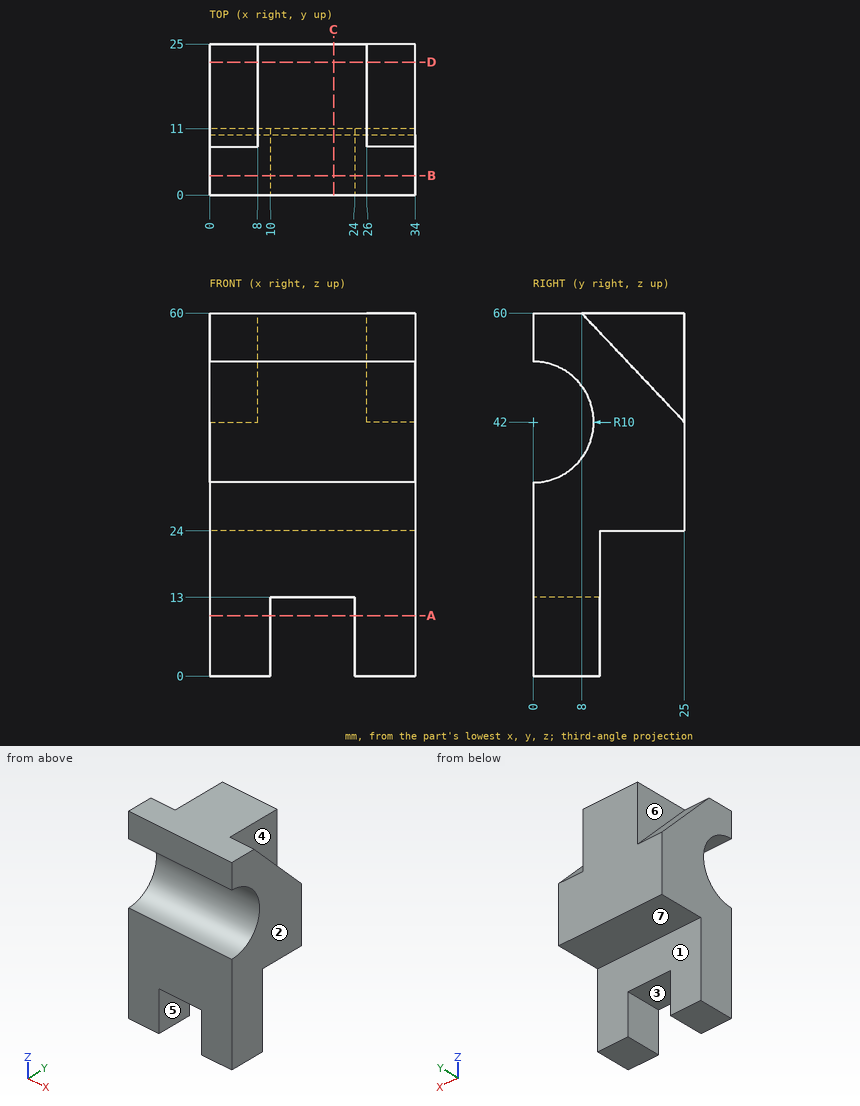
Study the drawing (mm; zero at the part's minimum x, y, z) and answer. A direction names the side the tool comes from. Coordinates: 2 decimals unless noted, no trailing zeros. Order: outer loops, then holes, each group sorted by start corner. A loop starts at its lowest first (then second) coordinate and runs counter-clockwise, first axis right, second up. Notation, with made-up numbers: (-14.75, 83) -> (6.25, 83) arc R24 ccw to (6.25, 101) -> close; hole circle Ø10 at (78.25, -32). An arc over 180 degrees is marked (long way). Answer in a Markdown table with one row per item. Add a question column.
Item 1: Which of the six approach directions +Z, -Z, +X, -X, +Y, -Y give full straight-line access (tool end or side, diameter ignored) to the marked faces 1, 2, 3 and 4?
Item 2: Find section B-B (y = 3.25). Write down the section's boundary in (x, z), then the cut area to 3 significant figures.
Item 3: Each of these flat-tipped pins is pushed along its axis until it touches: P1, Ø5, axis at x = 12, z = 47, coming from the -Y side; P2, Ø7, axis at x = 20, y = 21, coming from the -Z side; P3, Ø2, axis at x = 4.5, z = 10.5, coming from the +Y side. Where does it stop, or does it pass through?
Item 4: Find section D-D (y = 22). Write down the section's boundary in (x, z).
Item 5: Determine the mould class of the marked faces 5, 6 and 7 for opening direction X: +X half, -X half, draft (parallel to the pull), parting line (faces both ways), or undercut.
Item 6: Find section A-A (z = 10). Write down the section's boundary in (x, y).
Item 7: Find the intervals of material crossed by L1, parallel to X at y = 6.5, z = 12; L2, parallel to Z at x = 15, y = 14.75; L3, parallel to Z at x = 5, y = 4.75, in increasing order. Write a range as from..to.
Item 8: Find section C-C (x = 20.5). Write down the section's boundary in (y, z), then the cut area to 3 significant figures.
Result set:
| question | item | result |
|---|---|---|
| 1 | face 1 | -Z, +X, -X, +Y |
| 1 | face 2 | +Z, -Z, +X, +Y, -Y |
| 1 | face 3 | -Z, +Y, -Y |
| 1 | face 4 | +Z, +X, +Y |
| 2 | outline | (0, 0) -> (10, 0) -> (10, 13) -> (24, 13) -> (24, 0) -> (34, 0) -> (34, 32.54) -> (0, 32.54) -> close; (0, 51.46) -> (34, 51.46) -> (34, 60) -> (0, 60) -> close |
| 2 | area | 1,210 mm² |
| 3 | P1 | stops at y = 6.61 |
| 3 | P2 | stops at z = 24 |
| 3 | P3 | stops at y = 11 |
| 4 | outline | (0, 24) -> (34, 24) -> (34, 45.18) -> (26, 45.18) -> (26, 60) -> (8, 60) -> (8, 45.18) -> (0, 45.18) -> close |
| 5 | face 5 | undercut |
| 5 | face 6 | -X half |
| 5 | face 7 | draft |
| 6 | outline | (0, 0) -> (10, 0) -> (10, 11) -> (0, 11) -> close; (24, 0) -> (34, 0) -> (34, 11) -> (24, 11) -> close |
| 7 | L1 | x = 0..10, 24..34 |
| 7 | L2 | z = 24..60 |
| 7 | L3 | z = 0..33.2, 50.8..60 |
| 8 | outline | (0, 13) -> (11, 13) -> (11, 24) -> (25, 24) -> (25, 60) -> (0, 60) -> (0, 52) arc R10 cw to (0, 32) -> close |
| 8 | area | 864 mm² |
